from build123d import *

# Parameters (mm, degrees)
SKETCH_1_W              = 110
SKETCH_1_H              = 77
EXTRUDE_1_DEPTH         = 8
SKETCH_2_W              = 110
SKETCH_2_H              = 8
EXTRUDE_3_DEPTH         = 43
SKETCH_4_OUTSIDE_W      = 140.198
SKETCH_4_OUTSIDE_H      = 73.198
CUT_EXTRUDE_1_DEPTH     = 43
HOLE_WIZARD_7_0_7_1_D   = 9
HOLE_WIZARD_5_5_5_5_2_D = 5.5
CHAMFER_1_SIZE          = 2


with BuildPart() as part:
    # 草图1 → 凸台-拉伸1 (new body)
    with BuildSketch(Plane.XY):
        Rectangle(SKETCH_1_W, SKETCH_1_H)
    extrude(amount=EXTRUDE_1_DEPTH)

    # 草图2 → 凸台-拉伸3 (add)
    with BuildSketch(Plane.XY):
        with Locations((0, 34.5)):
            Rectangle(SKETCH_2_W, SKETCH_2_H)
    extrude(amount=EXTRUDE_3_DEPTH)

    # 草图4 outside → 切除-拉伸1 (cut)
    with BuildSketch(Plane(origin=(0, 38.5, 0), x_dir=(1, 0, 0), z_dir=(0, 1, 0))):
        with Locations((0, -21.5)):
            Rectangle(SKETCH_4_OUTSIDE_W, SKETCH_4_OUTSIDE_H)
        Polygon((-55, 0), (55, 0), (55, -12.75), (15.74, -43), (-15.74, -43), (-55, -12.75), align=None, mode=Mode.SUBTRACT)
    extrude(amount=-CUT_EXTRUDE_1_DEPTH, mode=Mode.SUBTRACT)

    # Ø7.0 (7) 直径孔1 (through all)
    with Locations(Plane.XY.offset(8)):
        with Locations((-48, -31.5), (48, -31.5), (48, -1.5), (-48, -1.5)):
            Hole(HOLE_WIZARD_7_0_7_1_D / 2)

    # Ø5.5 (5.5) 直径孔2 (through all)
    with Locations(Plane(origin=(0, 38.5, 0), x_dir=(1, 0, 0), z_dir=(0, 1, 0))):
        with Locations((-12.990381057, -15.5), (12.990381057, -15.5), (0, -38)):
            Hole(HOLE_WIZARD_5_5_5_5_2_D / 2)

    # 倒角1
    chamfer_1_edges = [part.edges().sort_by_distance(p)[0] for p in [
        (55, -38.5, 4),
        (-55, -38.5, 4),
    ]]
    chamfer(chamfer_1_edges, length=CHAMFER_1_SIZE)


solid = part.part
Source: CAD feature listing. Evaluate the final solid. Frame: model axes, mm. A direction names the side the tool comes from. Round coordinates to 2 decimals unless told otherwise and drop trailing zeros. Loops run counter-clockwise (first coordinate to the right, second up) from the corner with the lowest first, then second, coordinate; pieces in that order, holes last. Notation, with made-up numbers: M 59.25,19 L 71.25,19 A15 cw 71.25,38 Z; hole C -3,80.5 d2. An arc over 180 degrees is marked long. Answer as CSV lines item,"result".
Q1. Cut plane B-B (y = -1.5). Return the cut outline in (x, z), plus the area to 3 significant figures.
Verdict:
outline,"M -55,0 L -52.5,0 L -52.5,8 L -55,8 Z; M -43.5,0 L 43.5,0 L 43.5,8 L -43.5,8 Z; M 52.5,0 L 55,0 L 55,8 L 52.5,8 Z"
area,"736 mm^2"
Q2. Cut plane C-C (z = 15.5). Return the cut outline in (x, y), plus the area to 3 significant figures.
Verdict:
outline,"M -51.43,30.5 L -15.74,30.5 L -15.74,38.5 L -51.43,38.5 Z; M -10.24,30.5 L 10.24,30.5 L 10.24,38.5 L -10.24,38.5 Z; M 15.74,30.5 L 51.43,30.5 L 51.43,38.5 L 15.74,38.5 Z"
area,"735 mm^2"
Q3. Reachability of faces 1 (the face through (-52.292, -0.148, 3.944)), 2 (the face through (-1, -4, 8)) from +Z, -Z, +X, -X, +Y, -Y: full face, straight path, thin tool, end or side. Return the list, or none.
Verdict:
face 1,"+Z, -Z"
face 2,"+Z, +X, -X, -Y"
Q4. Line query: line 1 along Y through (x, z) = (48, 5); line 2 along X through (y, z) = (-31, 5); line 3 along Y through (x, z) = (45, 15.5). Output: solid intervals per line, ascending.
Verdict:
line 1,"y = -38.5 to -36, -27 to -6, 3 to 38.5"
line 2,"x = -55 to -52.47, -43.53 to 43.53, 52.47 to 55"
line 3,"y = 30.5 to 38.5"
Q5. Cut plane D-D (x = -48). Return the cut outline in (y, z).
Verdict:
outline,"M -38.5,0 L -36,0 L -36,8 L -38.5,8 Z; M -27,0 L -6,0 L -6,8 L -27,8 Z; M 3,0 L 38.5,0 L 38.5,18.14 L 30.5,18.14 L 30.5,8 L 3,8 Z"
Q6. Contact query for flat-ended pins moving along their axis: pin 1 (2 mm diameter, centred on x = -25.5, z = 32, fed in from -Y); pin 2 (5.5 mm diameter, centred on x = 48, y = -31.5, fed in from +Z); pin 3 (12 mm diameter, centred on x = 24.5, y = -19, fed in from -Z); pin 4 (11.5 mm diameter, centred on x = -48, y = -1.5, fed in from +Z). Output: stop coordinate, or through.
Verdict:
pin 1,"stops at y = 30.5"
pin 2,"passes through"
pin 3,"stops at z = 0"
pin 4,"stops at z = 8"
Q7. Cut plane A-A (x = 0). Return the cut outline in (y, z).
Verdict:
outline,"M -38.5,0 L 38.5,0 L 38.5,35.25 L 30.5,35.25 L 30.5,8 L -38.5,8 Z; M 30.5,40.75 L 38.5,40.75 L 38.5,43 L 30.5,43 Z"
Q8. Pull-direction query (Z, two-part tool) for faces 3 (the face through (-1, 1, 0)), 4 (the face through (-15.613, 34.444, 14.674)), 5 (the face through (0.358, 34.444, 35.273)), 6 (the face through (-1, 30.5, 21)); classes: +Z half, -Z half, draft (parallel to the pull), parting line (faces both ways), or undercut.
Verdict:
face 3,"-Z half"
face 4,"undercut"
face 5,"undercut"
face 6,"draft"
